Geometry check sheet. Reference: the model listing, model coordinates, mm. Coordinates: 2 decimals unless noted, no trailing zeros. Write each loop counter-clockwise with the first axis right and the second up, starting at its lowest first coordinate (ties: lowest second). Pieces come first, ordered by that corner, then holes. Notation, with made-up numbers: (63.5, 24) -> (112.5, 24) arc R18 ccw to (112.5, 55) -> close; hole circle Ø8 at (4, 39). An arc over 180 degrees is marked (long way). Use a Markdown table: item, result.
```python
from build123d import *

# Parameters (mm, degrees)
SKETCH_1_W             = 80
SKETCH_1_H             = 125
EXTRUDE_1_DEPTH        = 14
SKETCH_2_R             = 15
CUT_EXTRUDE_1_DEPTH    = 7
SKETCH_3_R             = 12
CUT_EXTRUDE_2_DEPTH    = 149.573214275
CHAMFER_2_SIZE         = 0.5
HOLE_WIZARD_M8_1_D     = 6.8
HOLE_WIZARD_M8_1_DEPTH = 22.25
HOLE_WIZARD_M8_1_TIP   = 2.042926105
SKETCH_10_R            = 2.75
CUT_EXTRUDE_3_DEPTH    = 150.067098986


with BuildPart() as part:
    # 草图1 → 凸台-拉伸1 (new body)
    with BuildSketch(Plane.XY):
        with Locations((40, -62.5)):
            Rectangle(SKETCH_1_W, SKETCH_1_H)
    extrude(amount=EXTRUDE_1_DEPTH)

    # 草图2 → 切除-拉伸1 (cut)
    with BuildSketch(Plane.XY.offset(14)):
        with Locations((40, -60)):
            Circle(SKETCH_2_R)
    extrude(amount=-CUT_EXTRUDE_1_DEPTH, mode=Mode.SUBTRACT)

    # 草图3 → 切除-拉伸2 (cut, through all)
    with BuildSketch(Plane.XY.offset(7)):
        with Locations((40, -60)):
            Circle(SKETCH_3_R)
    extrude(amount=-CUT_EXTRUDE_2_DEPTH, mode=Mode.SUBTRACT)

    # 倒角2
    chamfer_2_edges = [part.edges().sort_by_distance(p)[0] for p in [
        (25, -60, 14),
    ]]
    chamfer(chamfer_2_edges, length=CHAMFER_2_SIZE)

    # M8 螺纹孔1
    with Locations(Plane(origin=(0, 0, 0), x_dir=(1, 0, 0), z_dir=(0, 1, 0))):
        with Locations((67.5, -7), (12.5, -7)):
            Hole(HOLE_WIZARD_M8_1_D / 2, depth=HOLE_WIZARD_M8_1_DEPTH)
            with Locations((0, 0, -(HOLE_WIZARD_M8_1_DEPTH + HOLE_WIZARD_M8_1_TIP / 2))):  # 118° drill point
                Cone(0, HOLE_WIZARD_M8_1_D / 2, HOLE_WIZARD_M8_1_TIP, mode=Mode.SUBTRACT)

    # 草图10 → 切除-拉伸3 (cut, through all)
    with BuildSketch(Plane(origin=(0, 0, 0), x_dir=(-1, 0, 0), z_dir=(0, 0, -1))):
        with Locations((-65, -120)):
            Circle(SKETCH_10_R)
        with Locations((-15, -120)):
            Circle(SKETCH_10_R)
    extrude(amount=-CUT_EXTRUDE_3_DEPTH, mode=Mode.SUBTRACT)


solid = part.part
```
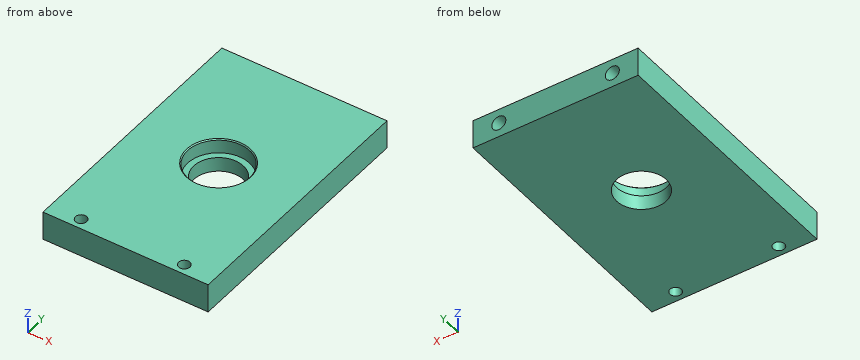
Item 1: Section check B-B on z = 1.75. Record the boundary of the cut face in (x, y), then the cut area to 3 significant figures.
Answer block:
| item | result |
|---|---|
| outline | (0, -125) -> (80, -125) -> (80, 0) -> (0, 0) -> close; hole circle Ø5.5 at (15, -120); hole circle Ø24 at (40, -60); hole circle Ø5.5 at (65, -120) |
| area | 9,500 mm^2 |
Item 2: Section check A-A on y = -60. Record the boundary of the cut face in (x, z).
Answer block:
| item | result |
|---|---|
| outline | (0, 0) -> (28, 0) -> (28, 7) -> (25, 7) -> (25, 13.5) -> (24.5, 14) -> (0, 14) -> close; (52, 0) -> (80, 0) -> (80, 14) -> (55.5, 14) -> (55, 13.5) -> (55, 7) -> (52, 7) -> close |
Item 3: Thickness scan on L1, parallel to Z at x = 67.5, y = -16; L2, parallel to Y at x = 40, z = 9; L3, parallel to Y at x = 40, z = 3. Record the ranges inside material, lowest first. Write a range as [from, to].
Answer block:
| item | result |
|---|---|
| L1 | z = [0, 3.6], [10.4, 14] |
| L2 | y = [-125, -75], [-45, 0] |
| L3 | y = [-125, -72], [-48, 0] |
Item 4: Depth check by flat-ended pin: P1, Ø8, axis at y = -67.5, z = 8.5, coming from the -X side; P2, Ø19, axis at x = 40, y = -60, coming from the +Z side; P3, Ø1, axis at x = 54, y = -65, coming from the +Z side; P4, Ø15, axis at x = 45, y = -58.5, coming from the +Z side. Enter the tip coordinate at first touch or a pass-through.
Answer block:
| item | result |
|---|---|
| P1 | stops at x = 0 |
| P2 | passes through |
| P3 | stops at z = 13.87 |
| P4 | stops at z = 7 |
